Can you work these out from the model? Positions are in its coordinate system, mm. A direction names the side the tool comes from. Give positions to 0.01 mm unless a question says otherwise; leave off trailing zeros. Order: outer loops, then holes, each group sorted by start corner. A loop starts at its lowest first (then second) coordinate and runs counter-clockwise, first axis right, second up. Notation, with made-up numbers: M 78.5,29 L 92.5,29 A20 ccw 92.5,68 Z; hole C 58.25,1.25 d10. An arc over 180 degrees is marked long. Use one line per item in the form item = value. Start each with the question number.
1. I need wall thicknesses on L1, parallel to X at y = 5.2, z = 0; L2, parallel to Z at x = -1, y = 3; L3, parallel to X at y = -4, z = 60. Which ranges of each line are inside material? Lowest first, please.
2. Will these pins go through, and if not, where does the flat tip stop? P1, Ø5, axis at x = 0, z = 0, coming from the +Y side; P2, Ø4.5, axis at x = 0, z = 60, coming from the -Y side.
3. We'd pull the mould along Z, two halves only. Please class faces 3 (the face through (0, 0, -75)), 4 (the face through (0, 4, -63)), 5 (the face through (-2, -6.25, 1)): +Z half, -Z half, draft (parallel to the pull), parting line (faces both ways), or undercut.
4. For faces 1 (the face through (-1, 1.75, 62)), 2 (the face through (-7.5, 0, 1)), which set-ups out of +Z, -Z, +X, -X, +Y, -Y let a thin tool reach every point of the face, with its end or its side?
5. I want a section at B-B, the plane y = -4.25. List the corners of the cut face in (x, z) for me, and give its area (3 significant figures).
6. I want a section at A-A, the plane z = -60. List the corners of the cut face in (x, y) for me.
```python
from build123d import *

# Parameters (mm, degrees)
SKETCH_1_W             = 15
SKETCH_1_H             = 12.5
EXTRUDE_1_DEPTH        = 75
SKETCH_2_R             = 3
CUT_EXTRUDE_1_DEPTH    = 4.5
SKETCH_3_R             = 2
CUT_EXTRUDE_2_DEPTH    = 77.40353395
PATTERN_LINEAR_1_COUNT = 6
PATTERN_LINEAR_1_PITCH = 60


with BuildPart() as part:
    # 草图1 → 凸台-拉伸1 (new, symmetric)
    with BuildSketch(Plane.XY):
        Rectangle(SKETCH_1_W, SKETCH_1_H)
    extrude(amount=EXTRUDE_1_DEPTH, both=True)

    # 草图2 → 切除-拉伸1 (cut)
    with BuildSketch(Plane(origin=(0, 6.25, 0), x_dir=(1, 0, 0), z_dir=(0, 1, 0))):
        with Locations(Location((0, -60, 0), (0, 0, 270))):
            Circle(SKETCH_2_R)
    cut_extrude_1 = extrude(amount=-CUT_EXTRUDE_1_DEPTH, mode=Mode.SUBTRACT)

    # 草图3 → 切除-拉伸2 (cut, through all)
    with BuildSketch(Plane(origin=(0, 6.25, 0), x_dir=(1, 0, 0), z_dir=(0, 1, 0))):
        with Locations(Location((0, -60, 0), (0, 0, 270))):
            Circle(SKETCH_3_R)
    cut_extrude_2 = extrude(amount=-CUT_EXTRUDE_2_DEPTH, mode=Mode.SUBTRACT)

    # 阵列(线性)1: 切除-拉伸1, 切除-拉伸2 ×6
    with Locations(*[(0, 0, -i * PATTERN_LINEAR_1_PITCH) for i in range(1, PATTERN_LINEAR_1_COUNT)]):
        add(cut_extrude_1, mode=Mode.SUBTRACT)
        add(cut_extrude_2, mode=Mode.SUBTRACT)


solid = part.part
```
Check result:
q1.L1 = -7.5 to -3, 3 to 7.5
q1.L2 = -75 to -62.83, -57.17 to -2.83, 2.83 to 57.17, 62.83 to 75
q1.L3 = -7.5 to -2, 2 to 7.5
q2.P1 = 1.75
q2.P2 = -6.25
q3.face_3 = -Z half
q3.face_4 = undercut
q3.face_5 = draft
q4.face_1 = +Y
q4.face_2 = +Z, -Z, -X, +Y, -Y
q5.outline = M -7.5,-75 L 7.5,-75 L 7.5,75 L -7.5,75 Z; hole C 0,-60 d4; hole C 0,0 d4; hole C 0,60 d4
q5.area = 2,210 mm2
q6.outline = M -7.5,-6.25 L -2,-6.25 L -2,1.75 L -3,1.75 L -3,6.25 L -7.5,6.25 Z; M 2,-6.25 L 7.5,-6.25 L 7.5,6.25 L 3,6.25 L 3,1.75 L 2,1.75 Z
